from build123d import *

# Parameters (mm, degrees)
FILLET1_R                                            = 1.6
HOLE_SIZE_PER_SOCKET_HEAD_CAP_SCREW_TYPE_D           = 11
HOLE_SIZE_PER_SOCKET_HEAD_CAP_SCREW_TYPE_CBORE_D     = 18
HOLE_SIZE_PER_SOCKET_HEAD_CAP_SCREW_TYPE_CBORE_DEPTH = 13
CIRPATTERN1_COUNT                                    = 12


with BuildPart() as part:
    # Sketch1 → Revolve1 (revolve)
    with BuildSketch(Plane.XY):
        Polygon((-149, 0), (-149, 16), (-194.5, 16), (-194.5, 7), (-177, 7), (-177, 0), align=None)
    revolve(axis=Axis((0, 32.824838348, 0), (0, -1, 0)))

    # Fillet1
    fillet1_edges = [part.edges().sort_by_distance(p)[0] for p in [
        (177, 7, 0),
    ]]
    fillet(fillet1_edges, radius=FILLET1_R)

    # Hole size per socket head cap screw type1 (through all)
    with Locations(Plane(origin=(0, 16, 0), x_dir=(-1, 0, 0), z_dir=(0, 1, 0))):
        with Locations((160, 0)):
            hole_size_per_socket_head_cap_screw_type = CounterBoreHole(HOLE_SIZE_PER_SOCKET_HEAD_CAP_SCREW_TYPE_D / 2, HOLE_SIZE_PER_SOCKET_HEAD_CAP_SCREW_TYPE_CBORE_D / 2, HOLE_SIZE_PER_SOCKET_HEAD_CAP_SCREW_TYPE_CBORE_DEPTH)

    # CirPattern1: Hole size per socket head cap screw type1 ×12 about axis
    cirpattern1_axis = Axis((0, 0, 0), (0, 1, 0))
    for i in range(1, CIRPATTERN1_COUNT):
        add(hole_size_per_socket_head_cap_screw_type.rotate(cirpattern1_axis, i * 360 / CIRPATTERN1_COUNT), mode=Mode.SUBTRACT)


solid = part.part
Check sheet for the modelled part. Datum: model origin and axes. Units: mm. A direction names the side the tool comes from. Round coordinates to 2 decimals unless told otherwise and drop trailing zeros. One line per item, written item: value.
(1) Release check for a two-part mould opening along X. For faces 1 (the face through (4, 3, -156)), 2 (the face through (-86, 7, 158)), 3 (the face through (38.37, 2.66, 172.79)) record: +X half, -X half, draft (parallel to the pull), parting line (faces both ways), or undercut.
Computed values:
face 1: undercut
face 2: draft
face 3: parting line
(2) Access from +Z, -Z, +X, -X, +Y, -Y to the whole of each face (thin tool, end or side, straight path). Record for faces 4 (the face through (-146.55, 9.59, -75.85)), 5 (the face through (140.67, 1.48, 85.08)).
Computed values:
face 4: +Y
face 5: +Y, -Y
(3) Sectioned sample at A-A, the plane z = 0. Count the separate pieces of the cut face and the enclosed holes in it, then the cut area to 3 significant figures.
Computed values:
separate pieces: 4
enclosed holes: 0
area: 678 mm^2
(4) Depth check by flat-ended pin: pin 1 Ø6.5 at (x, z) = (80, 138.56) entering from -Y; pin 2 Ø9 at (x, z) = (137.5, -77.5) entering from +Y; pin 3 Ø1.5 at (y, z) = (7.5, 77) entering from +X; pin 4 Ø6 at (y, z) = (9.5, 86.5) entering from +X. Enter the tip coordinate at first touch or a pass-through.
Computed values:
pin 1: passes through
pin 2: stops at y = 3
pin 3: stops at x = 178.93
pin 4: stops at x = 175.66
(5) Thickness scan on line 1 (Z direction, x = -80, y = 11); line 2 (X direction, y = 2.3, z = 80). Record the ranges inside material, lowest first.
Computed values:
line 1: z = -177.29 to -147.56, -129.56 to -125.7, 125.7 to 129.56, 147.56 to 177.29
line 2: x = -157.89 to -144.06, -133.06 to -125.7, 125.7 to 133.06, 144.06 to 157.89
